from build123d import *

# Parameters (mm, degrees)
EXTRUDE_1_DEPTH     = 375
SKETCH_2_R          = 6
EXTRUDE_2_DEPTH     = 70
EXTRUDE_START       = 11
SKETCH_3_R          = 6
EXTRUDE_3_DEPTH     = 11
FILLET_1_R          = 0.5
SKETCH_6_W          = 1
SKETCH_6_H          = 1.1
FILLET_2_R          = 0.5
SKETCH_7_W          = 10
SKETCH_7_H          = 2
CUT_EXTRUDE_1_DEPTH = 60


with BuildPart() as part:
    # 草图1 → 凸台-拉伸1 (new body)
    with BuildSketch(Plane.XY):
        Polygon((7, -4.041451884), (7, 4.041451884), (0, 8.082903769), (-7, 4.041451884), (-7, -4.041451884), (0, -8.082903769), align=None)
    extrude(amount=EXTRUDE_1_DEPTH)

    # 草图2 → 凸台-拉伸2 (add)
    with BuildSketch(Plane(origin=(0, 0, 0), x_dir=(-1, 0, 0), z_dir=(0, 0, -1))):
        with Locations(Location((0, 0, 0), (0, 0, 180))):
            Circle(SKETCH_2_R)
    extrude(amount=EXTRUDE_2_DEPTH)

    # 草图3 → 凸台-拉伸3 (add)
    with BuildSketch(Plane.XY.offset(375).offset(EXTRUDE_START)):
        Circle(SKETCH_3_R)
    extrude(amount=-EXTRUDE_3_DEPTH)

    # 圆角1
    fillet_1_edges = [part.edges().sort_by_distance(p)[0] for p in [
        (-6, 0, -70),
    ]]
    fillet(fillet_1_edges, radius=FILLET_1_R)

    # 草图6 → 切除-旋转2 (revolve, cut)
    with BuildSketch(Plane(origin=(0, 0, 0), x_dir=(1, 0, 0), z_dir=(0, 1, 0)), mode=Mode.PRIVATE) as cut_revolve_2_sk:
        with Locations((6, -383.55)):
            Rectangle(SKETCH_6_W, SKETCH_6_H)
    revolve(cut_revolve_2_sk.sketch.rotate(Axis((0, 0, 418.9281299), (0, 0, -1)), 180), axis=Axis((0, 0, 418.9281299), (0, 0, -1)), mode=Mode.SUBTRACT)

    # 圆角2
    fillet_2_edges = [part.edges().sort_by_distance(p)[0] for p in [
        (-6, 0, 386),
    ]]
    fillet(fillet_2_edges, radius=FILLET_2_R)

    # 草图7 → 切除-拉伸1 (cut)
    with BuildSketch(Plane(origin=(0, 0, -70), x_dir=(-1, 0, 0), z_dir=(0, 0, -1))):
        with Locations((0, 5.5)):
            Rectangle(SKETCH_7_W, SKETCH_7_H)
    extrude(amount=-CUT_EXTRUDE_1_DEPTH, mode=Mode.SUBTRACT)


solid = part.part
Can you work these out from the model? Positions are in its coordinate system, mm. A direction names the side the tool comes from. Coordinates: 2 decimals unless noted, no trailing zeros. Write each loop counter-clockwise with the first axis right and the second up, starting at its lowest first coordinate (ties: lowest second). Pieces come first, ordered by that corner, then holes. Notation, with made-up numbers: M 8,-26 L 36,-26 A35 ccw 36,6 Z; hole C -34.75,72 d2. An arc over 180 degrees is marked long. Use one line per item in the form item = value.
Q1. If we section it at B-B (z = 195.5): Write out the boundary of the cut face in (x, y).
Model answer:
outline = M -7,-4.04 L 0,-8.08 L 7,-4.04 L 7,4.04 L 0,8.08 L -7,4.04 Z
Q2. I need wall thicknesses on line 1 along Z through (x, y) = (-6, -1.5); line 2 along X through (y, z) = (0.75, -31); line 3 along Y through (x, z) = (2, 262). Which ranges of each line are inside material? Lowest first, please. Write a range as from..to.
Model answer:
line_1 = 0..375
line_2 = -5.95..5.95
line_3 = -6.93..6.93
Q3. For faces 1 (the flat face through (7, 0, 185)), 2 (the flat face through (0, 4.5, -40)), 3 (the cylindrical face through (-0.78, -5.95, -34.26)), 4 (the flat face through (3, -5, 384.1)), 5 (the cylindrical face through (-6, 0, 379)), which set-ups out of +Z, -Z, +X, -X, +Y, -Y let a thin tool reach every point of the face, with its end or its side?
Model answer:
face_1 = +Z, -Z, +X, +Y, -Y
face_2 = -Z, +X, -X, +Y
face_3 = -Z
face_4 = none
face_5 = +Z
Q4. We'd pull the mould along Z, two halves only. Please class faces 6 (the cylindrical face through (1.19, -5.37, 383.54)), 7 (the flat face through (-6, 2, 0)), 8 (the flat face through (0, 0, 386)): +Z half, -Z half, draft (parallel to the pull), parting line (faces both ways), or undercut.
Model answer:
face_6 = undercut
face_7 = -Z half
face_8 = +Z half
Q5. If we section it at C-C (z = -18.5): Write out the boundary of the cut face in (x, y), then the cut area to 3 significant figures.
Model answer:
outline = M -3.97,4.5 A6 ccw long 3.97,4.5 Z
area = 105 mm^2
Q6. If we section it at A-A (y = 0): Write out the boundary of the cut face in (x, z), then the cut area to 3 significant figures.
Model answer:
outline = M -7,0 L -6,0 L -6,-69.5 A0.5 ccw -5.5,-70 L 5.5,-70 A0.5 ccw 6,-69.5 L 6,0 L 7,0 L 7,375 L 6,375 L 6,383 L 5.5,383 L 5.5,384.1 L 6,384.1 L 6,385.5 A0.5 ccw 5.5,386 L -5.5,386 A0.5 ccw -6,385.5 L -6,384.1 L -5.5,384.1 L -5.5,383 L -6,383 L -6,375 L -7,375 Z
area = 6,220 mm^2
Q7. For P1, Ø2, axis at x = 4.5, y = 5, coming from the +Z side; P2, Ø6, axis at x = 3.5, z = 197, coming from the -Y side; P3, Ø0.8, axis at x = 2, y = 5.5, coming from the -Z side, each with a flat end and sliding along its axis, tell me the tip position at first contact or that it passes through.
Model answer:
P1 = 385.95
P2 = -7.79
P3 = -10
